from build123d import *

# Parameters (mm, degrees)
CHAMFER1_SIZE      = 1
SKETCH7_W          = 11.256792451
SKETCH7_H          = 6
CUT_EXTRUDE1_DEPTH = 10
SKETCH9_W          = 1.25
SKETCH9_H          = 21.5
CHAMFER2_SIZE      = 0.5
CIRPATTERN1_COUNT  = 4


with BuildPart() as part:
    # Sketch2 → Revolve1 (revolve)
    with BuildSketch(Plane(origin=(0, 0, 0), x_dir=(0, 0, -1), z_dir=(1, 0, 0)), mode=Mode.PRIVATE) as revolve1_sk:
        Polygon((8.5, 0), (21.5, 0), (21.5, 1), (11.5, 1), (11.5, 7), (8.5, 7), align=None)
    revolve(revolve1_sk.sketch.rotate(Axis((0, 67.294927727, 0), (0, -1, 0)), 180), axis=Axis((0, 67.294927727, 0), (0, -1, 0)))

    # Chamfer1
    chamfer1_edges = [part.edges().sort_by_distance(p)[0] for p in [
        (0, 0, -8.5),
    ]]
    chamfer(chamfer1_edges, length=CHAMFER1_SIZE)

    # Sketch7 → Cut-Extrude1 (cut)
    with BuildSketch(Plane(origin=(0, 1, 0), x_dir=(1, 0, 0), z_dir=(0, 1, 0))):
        with Locations((18.128396226, 0)):
            Rectangle(SKETCH7_W, SKETCH7_H)
    extrude(amount=-CUT_EXTRUDE1_DEPTH, mode=Mode.SUBTRACT)

    # Sketch9 → M3 Tapped Hole2 (revolve, cut)
    with BuildSketch(Plane(origin=(0, 4, 0), x_dir=(0, 0, -1), z_dir=(0, 1, 0))):
        with Locations((0.625, 10.75)):
            Rectangle(SKETCH9_W, SKETCH9_H)
    m3_tapped_hole2 = revolve(axis=Axis((6.35, 4, 0), (-1, 0, 0)), mode=Mode.SUBTRACT)

    # Chamfer2
    chamfer2_edges = [part.edges().sort_by_distance(p)[0] for p in [
        (0, 7, -11.5),
    ]]
    chamfer(chamfer2_edges, length=CHAMFER2_SIZE)

    # CirPattern1: M3 Tapped Hole2 ×4 about axis, 1 skipped
    cirpattern1_axis = Axis((0, 67.294927727, 0), (0, 1, 0))
    add([m3_tapped_hole2.rotate(cirpattern1_axis, i * 360 / CIRPATTERN1_COUNT) for i in range(1, CIRPATTERN1_COUNT) if i not in (2,)], mode=Mode.SUBTRACT)


solid = part.part
For this review, take the finished solid that the model builds, in its own axes (mm). A direction names the side the tool comes from. Round coordinates to 2 decimals unless told otherwise and drop trailing zeros. Loops run counter-clockwise (first coordinate to the right, second up) from the corner with the lowest first, then second, coordinate; pieces in that order, holes last. Notation, with made-up numbers: (78, 89) - (88, 89) arc R18 ccw to (88, 99) - close; hole circle Ø1 at (-35.75, -33.5). An arc over 180 degrees is marked (long way). Use one line per item in the form item = value.
1) Clearance check with flat-ended pins moving along their axes: P1, Ø0.8, axis at x = 17, y = 0.5, coming from the -Z side; P2, Ø2, axis at y = 4, z = 1, coming from the -X side; P3, Ø1.1, axis at x = 19, y = 0.5, coming from the +Z side; P4, Ø10, axis at x = 0, z = 0, coming from the +Y side. State where each tip first meets the part, or that it passes through.
Solutions:
P1 = -13.66
P2 = -11.47
P3 = 11.04
P4 = through
2) Wall thickness on probe 1 along X at (y, z) = (2.5, 0); probe 2 along Y at (x, z) = (-9.75, 0); probe 3 along Y at (x, z) = (16.5, -9.5): over which ranges is each line inside the solid? List them lowest first.
Solutions:
probe_1 = -11.5 to -8.5, 8.5 to 11.5
probe_2 = 0 to 2.75, 5.25 to 7
probe_3 = 0 to 1
3) We need section D-D on z = 14. Write out the cut boundary in (x, y), then the cut area to 3 significant figures.
Solutions:
outline = (-16.32, 0) - (16.32, 0) - (16.32, 1) - (-16.32, 1) - close
area = 32.6 mm2
4) We need section A-A on z = 0. Write out the cut boundary in (x, y), then the cut area to 4 significant figures.
Solutions:
outline = (-21.5, 0) - (-9.5, 0) - (-8.5, 1) - (-8.5, 2.75) - (-11.5, 2.75) - (-11.5, 1) - (-21.5, 1) - close; (-11.5, 5.25) - (-8.5, 5.25) - (-8.5, 7) - (-11, 7) - (-11.5, 6.5) - close; (8.5, 1) - (9.5, 0) - (12.5, 0) - (12.5, 1) - (11.5, 1) - (11.5, 6.5) - (11, 7) - (8.5, 7) - close
area = 44.25 mm2
5) We need section B-B on x = 0. Write out the cut boundary in (y, z).
Solutions:
outline = (0, -21.5) - (1, -21.5) - (1, -11.5) - (2.75, -11.5) - (2.75, -8.5) - (1, -8.5) - (0, -9.5) - close; (0, 9.5) - (1, 8.5) - (2.75, 8.5) - (2.75, 11.5) - (1, 11.5) - (1, 21.5) - (0, 21.5) - close; (5.25, -11.5) - (6.5, -11.5) - (7, -11) - (7, -8.5) - (5.25, -8.5) - close; (5.25, 8.5) - (7, 8.5) - (7, 11) - (6.5, 11.5) - (5.25, 11.5) - close
6) Mouldability with a two-part tool opening along X and no side actions: class faces 4 (the face through (-9.97, 5.22, 0.27)), 5 (the face through (3.26, 3.96, 7.85)), 6 (the face through (-3.45, 3.79, 10.97)) as pulls with the +X half, pulls with the -X half, needs draft (parallel to the pull), parting line crosses it, or undercut.
Solutions:
face_4 = needs draft
face_5 = undercut
face_6 = parting line crosses it
7) Tool access review of faces 1 (the face through (16.8, 0.5, 3)), 2 (the face through (9, 1, 9)), 3 (the face through (-21.48, 0.51, 0.9)): name each direction out of +Z, -Z, +X, -X, +Y, -Y from which nothing blocks a thin tool from reaching the whole face with its end or side.
Solutions:
face_1 = +X, +Y, -Y
face_2 = +Y
face_3 = +Y, -Y
8) We need section C-C on y = 4. Write out the cut boundary in (x, z).
Solutions:
outline = (-11.43, -1.25) arc R11.5 ccw to (-1.25, -11.43) - (-1.25, -8.41) arc R8.5 cw to (-8.41, -1.25) - close; (-11.43, 1.25) - (-8.41, 1.25) arc R8.5 cw to (-1.25, 8.41) - (-1.25, 11.43) arc R11.5 ccw to start; (1.25, -11.43) arc R11.5 ccw to (1.25, 11.43) - (1.25, 8.41) arc R8.5 cw to (1.25, -8.41) - close
